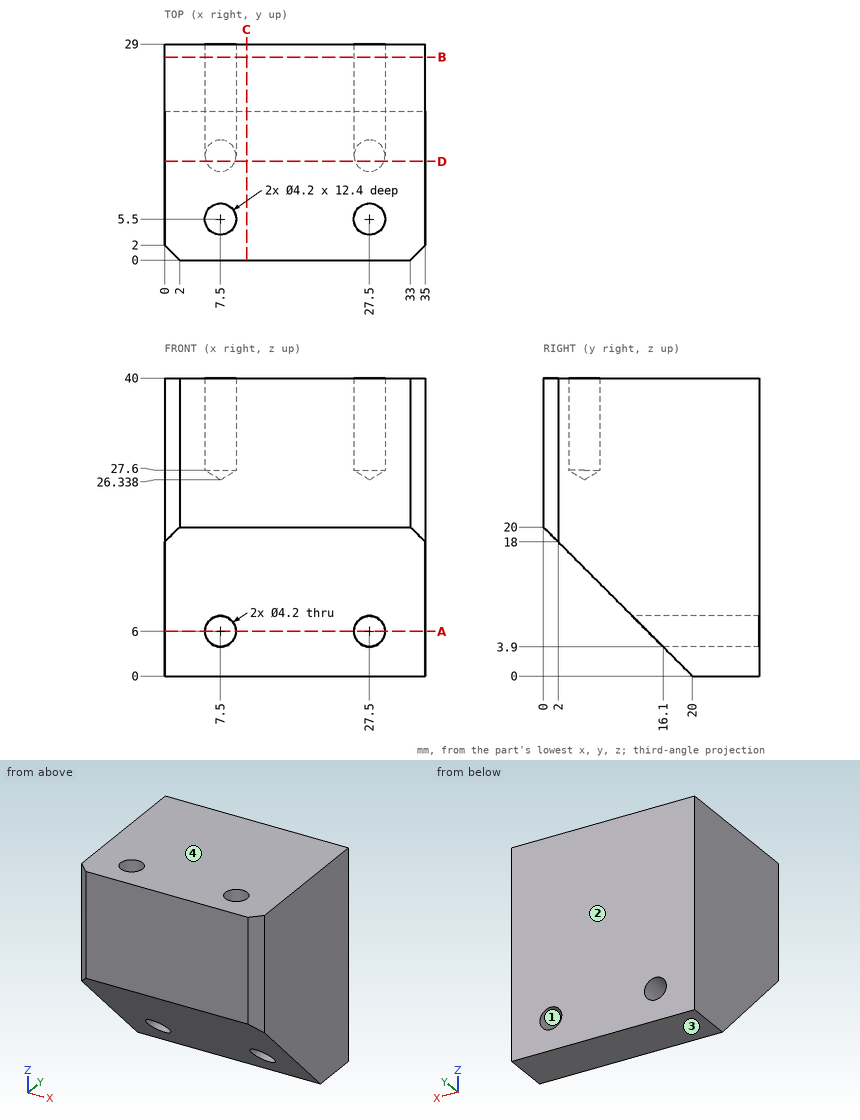
Geometry: see drawing. Coordinates: mm, zero at the bounding-box minimum. Coordinates: 2 decimals unless noted, no trailing zeros. Loops run counter-clockwise (first coordinate to the right, second up) from the corner with the lowest first, then second, coordinate; pieces in that order, holes last. Notation, with made-up numbers: (57, 83.5) -> (108, 83.5) arc R16 ccw to (108, 114.5) -> close; hole circle Ø5 at (55, 25). An arc over 180 degrees is marked (long way). Write item = value, one per line. Start each with the question number.
Item 1: Cut plane A-A, the plane z = 6. Return loops of the section in (x, y).
Item 2: Cut plane B-B, the plane y = 27.25. Return loops of the section in (x, z), plus the area to 3 significant figures.
Item 3: Cut plane C-C, the plane x = 11. Return loops of the section in (y, z).
Item 4: Material intervals for line 1 (X direction, y = 5.5, z = 34.75); line 2 (X direction, y = 4.5, z = 35); line 3 (Y direction, x = 7, z = 37), sorted ascending.
Item 5: First-contact query: P1, Ø2.5, axis at x = 7.5, y = 5.5, coming from the -Z side; P2, Ø6.5, axis at x = 7.5, z = 6, coming from the -Y side; P3, Ø5.5, axis at x = 27.5, y = 5.5, coming from the -Z side. Flat tips, straight axial feed; report the tip coordinate or a pass-through.
Item 6: Cut plane D-D, the plane y = 13.25. Return loops of the section in (x, z).
Item 7: Mould query, pull axis Z, two halves, no side actions, for the marked faces 1, 2, 3 and 4. Classes: pulls with the +Z half, pulls with the -Z half, needs draft (parallel to the pull), parting line crosses it, or undercut.
Ans:
q1.outline = (0, 14) -> (5.4, 14) -> (5.4, 29) -> (0, 29) -> close; (9.6, 14) -> (25.4, 14) -> (25.4, 29) -> (9.6, 29) -> close; (29.6, 14) -> (35, 14) -> (35, 29) -> (29.6, 29) -> close
q2.outline = (0, 0) -> (35, 0) -> (35, 40) -> (0, 40) -> close; hole circle Ø4.2 at (7.5, 6); hole circle Ø4.2 at (27.5, 6)
q2.area = 1,370 mm²
q3.outline = (0, 20) -> (20, 0) -> (29, 0) -> (29, 40) -> (0, 40) -> close
q4.line_1 = 0 to 5.4, 9.6 to 25.4, 29.6 to 35
q4.line_2 = 0 to 5.65, 9.35 to 25.65, 29.35 to 35
q4.line_3 = 0 to 3.46, 7.54 to 29
q5.P1 = 13.25
q5.P2 = 10.75
q5.P3 = 11.75
q6.outline = (0, 6.75) -> (5.54, 6.75) arc R2.1 cw to (9.46, 6.75) -> (25.54, 6.75) arc R2.1 cw to (29.46, 6.75) -> (35, 6.75) -> (35, 40) -> (0, 40) -> close
q7.face_1 = undercut
q7.face_2 = needs draft
q7.face_3 = pulls with the -Z half
q7.face_4 = pulls with the +Z half
